Verification items for the finished model (mm, model axes). A direction names the side the tool comes from. Give positions to 0.01 mm unless a question says otherwise; leave off trailing zeros. Loops run counter-clockwise (first coordinate to the right, second up) from the corner with the lowest first, then second, coordinate; pieces in that order, holes last. Notation, with made-up numbers: (25.5, 48.25) - (58.5, 48.25) arc R13 ccw to (58.5, 72.25) - close; hole circle Ø11 at (18.5, 76). An arc over 180 degrees is marked (long way). Use one line per item in the form item = value.
```python
from build123d import *

# Parameters (mm, degrees)
SKETCH1_R           = 7
SKETCH1_R_2         = 4.5
BOSS_EXTRUDE1_DEPTH = 30
SKETCH2_W           = 15
SKETCH2_H           = 22
CUT_EXTRUDE1_DEPTH  = 59.976690311
CHAMFER1_SIZE       = 2
SKETCH3_R           = 10
CUT_EXTRUDE2_DEPTH  = 5
SKETCH4_W           = 5
SKETCH4_H           = 10
BOSS_EXTRUDE2_DEPTH = 4
CUT_EXTRUDE3_DEPTH  = 12


with BuildPart() as part:
    # Sketch1 → Boss-Extrude1 (new body)
    with BuildSketch(Plane.XY):
        Polygon((-21.5, 23), (-0.5, 23), (-0.5, 14), (21.5, 14), (21.5, -14), (-0.5, -14), (-0.5, -23), (-21.5, -23), align=None)
        with Locations((7.5, 0)):
            Circle(SKETCH1_R, mode=Mode.SUBTRACT)
        with Locations((-14.5, 15)):
            Circle(SKETCH1_R_2, mode=Mode.SUBTRACT)
        with Locations((-14.5, -15)):
            Circle(SKETCH1_R_2, mode=Mode.SUBTRACT)
    extrude(amount=BOSS_EXTRUDE1_DEPTH)

    # Sketch2 → Cut-Extrude1 (cut, through all)
    with BuildSketch(Plane(origin=(0, 23, 0), x_dir=(1, 0, 0), z_dir=(0, 1, 0))):
        with Locations((-14, -19)):
            Rectangle(SKETCH2_W, SKETCH2_H)
    extrude(amount=-CUT_EXTRUDE1_DEPTH, mode=Mode.SUBTRACT)

    # Chamfer1
    chamfer1_edges = [part.edges().sort_by_distance(p)[0] for p in [
        (21.5, 14, 15),
        (21.5, -14, 15),
    ]]
    chamfer(chamfer1_edges, length=CHAMFER1_SIZE)

    # Sketch3 → Cut-Extrude2 (cut)
    with BuildSketch(Plane.XY.offset(30)):
        with Locations((7.5, 0)):
            Circle(SKETCH3_R)
    extrude(amount=-CUT_EXTRUDE2_DEPTH, mode=Mode.SUBTRACT)

    # Sketch4 → Boss-Extrude2 (add)
    with BuildSketch(Plane.XY.offset(8)):
        with Locations((-19, 0)):
            Rectangle(SKETCH4_W, SKETCH4_H)
    extrude(amount=BOSS_EXTRUDE2_DEPTH)

    # Sketch5 → Cut-Extrude3 (cut)
    with BuildSketch(Plane(origin=(21.5, 0, 0), x_dir=(0, 0, -1), z_dir=(1, 0, 0))):
        with BuildLine():
            Line((-19, 4), (-11, 4))
            ThreePointArc((-11, 4), (-7, 0), (-11, -4))
            Line((-11, -4), (-19, -4))
            ThreePointArc((-19, -4), (-23, 0), (-19, 4))
        make_face()
    extrude(amount=-CUT_EXTRUDE3_DEPTH, mode=Mode.SUBTRACT)


solid = part.part
```
1. Depth check by flat-ended pin: pin 1 Ø3 at (x, z) = (-16, 8.5) entering from +Y; pin 2 Ø2 at (y, z) = (13, 21) entering from -X; pin 3 Ø4 at (x, z) = (18.5, 17) entering from -Y; pin 4 Ø4.5 at (x, z) = (-19, 11) entering from -Y. Enter the tip coordinate at first touch or a pass-through.
Result set:
pin_1 = 23
pin_2 = -6.5
pin_3 = -14
pin_4 = -5
2. Section check B-B, the plane x = -14.5. Record the cut outline in (y, z).
Result set:
outline = (-23, 0) - (-19.5, 0) - (-19.5, 8) - (-23, 8) - close; (-10.5, 0) - (10.5, 0) - (10.5, 8) - (-10.5, 8) - close; (19.5, 0) - (23, 0) - (23, 8) - (19.5, 8) - close
3. Section check D-D, the plane x = 7.5. Record the cut outline in (y, z), then the cut area to 3 significant figures.
Result set:
outline = (-14, 0) - (-7, 0) - (-7, 25) - (-10, 25) - (-10, 30) - (-14, 30) - close; (7, 0) - (14, 0) - (14, 30) - (10, 30) - (10, 25) - (7, 25) - close
area = 390 mm²
4. Tool access check on faces 5 (the flat face through (-19, 5, 10)), 6 (the flat face through (-0.5, 19, 15)), 7 (the flat face through (-16.5, 0, 10)), 8 (the flat face through (-19, -5, 10)). Record the directions out of +Z, -Z, +X, -X, +Y, -Y that give a thin tool (end or side, any length) a straight path to the whole face; none if there is none.
Result set:
face_5 = +Z, -X, +Y
face_6 = +Z, -Z, +X, +Y
face_7 = +Z, +Y, -Y
face_8 = +Z, -X, -Y
5. Scan lines: probe 1 along Y at (x, z) = (-14.5, 3); probe 2 along X at (y, z) = (0, 11.75); probe 3 along X at (y, z) = (-15, 5). Record each from-to range of solid material in increasing order.
Result set:
probe_1 = -23 to -19.5, -10.5 to 10.5, 19.5 to 23
probe_2 = -21.5 to -16.5, -6.5 to 0.5
probe_3 = -21.5 to -19, -10 to -0.5
6. Section check A-A, the plane z = 3. Record the cut outline in (x, y), then the cut area to 3 significant figures.
Result set:
outline = (-21.5, -23) - (-0.5, -23) - (-0.5, -14) - (19.5, -14) - (21.5, -12) - (21.5, 12) - (19.5, 14) - (-0.5, 14) - (-0.5, 23) - (-21.5, 23) - close; hole circle Ø9 at (-14.5, -15); hole circle Ø9 at (-14.5, 15); hole circle Ø14 at (7.5, 0)
area = 1,300 mm²
7. Draft check along Y on faces 1 (the flat face through (10, 7, 25)), 2 (the flat face through (21.5, 6, 15)), 3 (the cylindrical face through (17, 0, 7)), 4 (the flat face through (9, 14, 15)). Enter one of: released by +Y, released by -Y, zero draft, split by the parting line, or undercut.
Result set:
face_1 = undercut
face_2 = zero draft
face_3 = undercut
face_4 = released by +Y
8. Section check C-C, the plane y = 15. Record the cut outline in (x, z).
Result set:
outline = (-21.5, 0) - (-19, 0) - (-19, 8) - (-21.5, 8) - close; (-10, 0) - (-0.5, 0) - (-0.5, 30) - (-6.5, 30) - (-6.5, 8) - (-10, 8) - close
